Geometry: final body of the model. Coordinates: model frame, mm. A direction names the side the tool comes from. Coordinates: 2 decimals unless noted, no trailing zeros. Order: outer loops, then holes, each group sorted by start corner. A loop starts at its lowest first (then second) coordinate and runs counter-clockwise, first axis right, second up. Notation, with made-up numbers: (1, 16) -> (23, 16) arc R23 ccw to (23, 43) -> close; hole circle Ø6 at (73, 45.5). An arc over 180 degrees is marked (long way). Use one line per item in the form item = value.
```python
from build123d import *

# Parameters (mm, degrees)
SKETCH1_R                     = 33
BOSS_EXTRUDE1_DEPTH           = 22.5
SKETCH2_R                     = 29
BOSS_EXTRUDE2_DEPTH           = 1.5
SKETCH3_R                     = 20
CUT_EXTRUDE1_DEPTH            = 58.5
M3_TAPPED_HOLE1_D             = 2.5
M3_TAPPED_HOLE1_DEPTH         = 7.5
M3_TAPPED_HOLE1_CSINK_D       = 3.05
M3_TAPPED_HOLE1_CSINK_ANGLE   = 90
M3_TAPPED_HOLE1_TIP           = 0.751075774
SKETCH7_R                     = 2
CUT_EXTRUDE2_DEPTH            = 5
SKETCH8_R                     = 21
CUT_EXTRUDE3_DEPTH            = 1.5
SKETCH9_R                     = 29
CUT_EXTRUDE4_DEPTH            = 0.36
SKETCH10_R                    = 21.75
CUT_EXTRUDE5_DEPTH            = 7.2
M1_6_TAPPED_HOLE1_D           = 1.25
M1_6_TAPPED_HOLE1_DEPTH       = 4.25
M1_6_TAPPED_HOLE1_CSINK_D     = 1.65
M1_6_TAPPED_HOLE1_CSINK_ANGLE = 90
M1_6_TAPPED_HOLE1_TIP         = 0.375537887
CUT_EXTRUDE6_DEPTH            = 3


with BuildPart() as part:
    # Sketch1 → Boss-Extrude1 (new body)
    with BuildSketch(Plane(origin=(0, 0, 0), x_dir=(1, 0, 0), z_dir=(0, 1, 0))):
        with Locations(Location((0, 0, 0), (0, 0, 90))):
            Circle(SKETCH1_R)
    extrude(amount=BOSS_EXTRUDE1_DEPTH)

    # Sketch2 → Boss-Extrude2 (add)
    with BuildSketch(Plane(origin=(0, 22.5, 0), x_dir=(1, 0, 0), z_dir=(0, 1, 0))):
        with Locations(Location((0, 0, 0), (0, 0, 270))):
            Circle(SKETCH2_R)
    extrude(amount=BOSS_EXTRUDE2_DEPTH)

    # Sketch3 → Cut-Extrude1 (cut)
    with BuildSketch(Plane(origin=(0, 24, 0), x_dir=(1, 0, 0), z_dir=(0, 1, 0))):
        with Locations(Location((0, 0, 0), (0, 0, 270))):
            Circle(SKETCH3_R)
    extrude(amount=-CUT_EXTRUDE1_DEPTH, mode=Mode.SUBTRACT)

    # M3 Tapped Hole1
    with Locations(Plane(origin=(0, 24, 0), x_dir=(1, 0, 0), z_dir=(0, 1, 0))):
        with Locations((25, 0), (0, 25), (-25, 0), (0, -25)):
            CounterSinkHole(M3_TAPPED_HOLE1_D / 2, M3_TAPPED_HOLE1_CSINK_D / 2, depth=M3_TAPPED_HOLE1_DEPTH, counter_sink_angle=M3_TAPPED_HOLE1_CSINK_ANGLE)
            with Locations((0, 0, -(M3_TAPPED_HOLE1_DEPTH + M3_TAPPED_HOLE1_TIP / 2))):  # 118° drill point
                Cone(0, M3_TAPPED_HOLE1_D / 2, M3_TAPPED_HOLE1_TIP, mode=Mode.SUBTRACT)

    # Sketch7 → Cut-Extrude2 (cut)
    with BuildSketch(Plane(origin=(0, 24, 0), x_dir=(1, 0, 0), z_dir=(0, 1, 0))):
        with Locations(Location((-17.67766953, 17.67766953, 0), (0, 0, 270))):
            Circle(SKETCH7_R)
        with Locations(Location((17.67766953, -17.67766953, 0), (0, 0, 270))):
            Circle(SKETCH7_R)
    extrude(amount=-CUT_EXTRUDE2_DEPTH, mode=Mode.SUBTRACT)

    # Sketch8 → Cut-Extrude3 (cut)
    with BuildSketch(Plane(origin=(0, 24, 0), x_dir=(1, 0, 0), z_dir=(0, 1, 0))):
        with Locations(Location((0, 0, 0), (0, 0, 270))):
            Circle(SKETCH8_R)
    extrude(amount=-CUT_EXTRUDE3_DEPTH, mode=Mode.SUBTRACT)

    # Sketch9 → Cut-Extrude4 (cut)
    with BuildSketch(Plane.XZ):
        with Locations(Location((0, 0, 0), (0, 0, 90))):
            Circle(SKETCH9_R)
    extrude(amount=-CUT_EXTRUDE4_DEPTH, mode=Mode.SUBTRACT)

    # Sketch10 → Cut-Extrude5 (cut)
    with BuildSketch(Plane.XZ.offset(-0.36)):
        with Locations(Location((0, 0, 0), (0, 0, 270))):
            Circle(SKETCH10_R)
    extrude(amount=-CUT_EXTRUDE5_DEPTH, mode=Mode.SUBTRACT)

    # M1.6 Tapped Hole1
    with Locations(Plane(origin=(0, 0, 0), x_dir=(-1, 0, 0), z_dir=(0, -1, 0))):
        with Locations((0, 0), (0, 31), (26.846787517, 15.5), (26.846787517, -15.5), (0, -31), (-26.846787517, -15.5), (-26.846787517, 15.5)):
            CounterSinkHole(M1_6_TAPPED_HOLE1_D / 2, M1_6_TAPPED_HOLE1_CSINK_D / 2, depth=M1_6_TAPPED_HOLE1_DEPTH, counter_sink_angle=M1_6_TAPPED_HOLE1_CSINK_ANGLE)
            with Locations((0, 0, -(M1_6_TAPPED_HOLE1_DEPTH + M1_6_TAPPED_HOLE1_TIP / 2))):  # 118° drill point
                Cone(0, M1_6_TAPPED_HOLE1_D / 2, M1_6_TAPPED_HOLE1_TIP, mode=Mode.SUBTRACT)

    # Sketch15 → Cut-Extrude6 (cut)
    with BuildSketch(Plane.XZ):
        Polygon((19.632226772, 24.641961986), (12.362677286, 29.333923153), (15.170555531, 33.68434489), (22.766930333, 28.781441946), align=None)
    extrude(amount=-CUT_EXTRUDE6_DEPTH, mode=Mode.SUBTRACT)


solid = part.part
```
1) Section C-C, the plane y = 13.5. Output: boundary loops of the cut face in (x, z).
Results found:
outline = circle Ø66 at (0, 0); hole circle Ø40 at (0, 0)
2) Section B-B, the plane y = 21.5. Output: boundary loops of the cut face in (x, z).
Results found:
outline = circle Ø66 at (0, 0); hole circle Ø2.5 at (-25, 0); hole circle Ø40 at (0, 0); hole circle Ø4 at (-17.68, -17.68); hole circle Ø2.5 at (0, -25); hole circle Ø2.5 at (0, 25); hole circle Ø4 at (17.68, 17.68); hole circle Ø2.5 at (25, 0)
3) Section A-A, the plane z = -9.5. Output: boundary loops of the cut face in (x, y), and give its area (3 significant figures).
Results found:
outline = (-31.6, 0) -> (-27.4, 0) -> (-27.4, 0.36) -> (-19.57, 0.36) -> (-19.57, 7.56) -> (-17.6, 7.56) -> (-17.6, 22.5) -> (-18.73, 22.5) -> (-18.73, 24) -> (-27.4, 24) -> (-27.4, 22.5) -> (-31.6, 22.5) -> close; (17.6, 7.56) -> (19.57, 7.56) -> (19.57, 0.36) -> (27.4, 0.36) -> (27.4, 0) -> (31.6, 0) -> (31.6, 22.5) -> (27.4, 22.5) -> (27.4, 24) -> (18.73, 24) -> (18.73, 22.5) -> (17.6, 22.5) -> close
area = 621 mm2
4) Pull-direction query (X, two-part tool) for faces 4 (the conical face through (25.2, 15.88, 0.08)), 5 (the flat face through (-15, 24, 15)); classes: released by +X, released by -X, zero draft, split by the parting line, or undercut.
Results found:
face_4 = undercut
face_5 = zero draft
5) Contact query for flat-ended pins moving along their axis: P1, Ø8, axis at y = 15, z = -9.5, coming from the -X side; P2, Ø4, axis at x = 25, z = 0, coming from the -Y side; P3, Ø0.8, axis at x = 0, z = 31, coming from the -Y side. Output: stop coordinate, or through.
Results found:
P1 = -32.54
P2 = 0.36
P3 = 4.39
6) Material intervals for probe 1 along X at (y, z) = (0.1, 0); probe 2 along X at (y, z) = (3.25, 0); probe 3 along Z at (x, y) = (-27, 2.5), sorted ascending. Write a range as from..to.
Results found:
probe_1 = -33..-29, 29..33
probe_2 = -33..-21.75, 21.75..33
probe_3 = -18.97..-16.11, -14.89..14.89, 16.11..18.97
7) Section D-D, the plane z = 2.5. Output: boundary loops of the cut face in (x, y), and give its area (3 significant figures).
Results found:
outline = (-32.91, 0) -> (-28.89, 0) -> (-28.89, 0.36) -> (-21.61, 0.36) -> (-21.61, 7.56) -> (-19.84, 7.56) -> (-19.84, 22.5) -> (-20.85, 22.5) -> (-20.85, 24) -> (-28.89, 24) -> (-28.89, 22.5) -> (-32.91, 22.5) -> close; (19.84, 7.56) -> (21.61, 7.56) -> (21.61, 0.36) -> (28.89, 0.36) -> (28.89, 0) -> (32.91, 0) -> (32.91, 22.5) -> (28.89, 22.5) -> (28.89, 24) -> (20.85, 24) -> (20.85, 22.5) -> (19.84, 22.5) -> close
area = 580 mm2
8) Access query for faces 1 (the cylindrical face through (11.107, 0.177, 26.789)), 2 (the cylindrical face through (-19.524, 15.135, -4.336)), 3 (the flat face through (-18, 19, -18)). Directions: +Z, -Z, +X, -X, +Y, -Y. A direction counts if a zero-diameter tool reaches every point of the face in a straight line with its end or side. Return the directions, or none.
Results found:
face_1 = -Y
face_2 = +Y, -Y
face_3 = +Y
